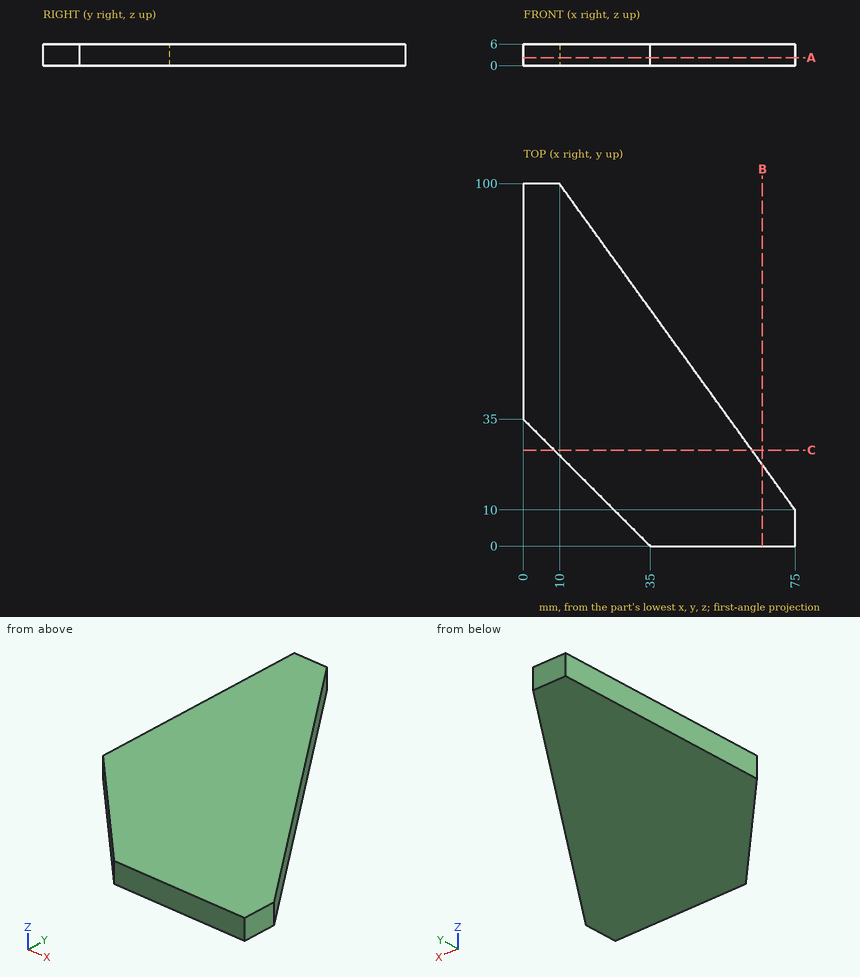
Could you check a few things on this drawing? It's one solid part, dimensions in mm from its lowest x, y, z. Round coordinates to 2 decimals unless told otherwise and drop trailing zeros. Loops run counter-clockwise (first coordinate to the right, second up) from the corner with the lowest first, then second, coordinate; pieces in that order, holes last. Notation, with made-up numbers: M -0.75,57 L 20.25,57 A28 cw 20.25,86 Z; hole C 1.5,84.25 d4. An arc over 180 degrees is marked long. Write each question's results on one line, items separated by ' | '. Start each with the question number.
(1) I want a section at A-A (z = 2.25). Please give me the cut outline in (x, y), then the cut area to 3 significant figures.
(2) Will these pins go through, and if not, where does the flat tip stop? P1, Ø2, axis at x = 30, z = 5, coming from the +Y side; P2, Ø3, axis at x = 25.5, y = 67.5, coming from the -Z side; P3, Ø1, axis at y = 83, z = 3.5, coming from the +X side; P4, Ø1.5, axis at x = 11, z = 0.5, coming from the +Y side.
(3) I want a section at C-C (y = 26.5). Please give me the cut outline in (x, z), then the cut area to 4 significant figures.
(4) If I drill on probe 1 along Y at (x, z) = (55, 2.25); probe 2 along X at (y, z) = (68, 2.5); probe 3 along X at (y, z) = (16, 4.5), over which ranges is the centre line in solid material (lowest first)? Write a range as from..to.
(5) I want a section at B-B (x = 66). Please give me the cut outline in (y, z), then the cut area to 3 significant figures.
Solved:
1) outline: M 0,35 L 35,0 L 75,0 L 75,10 L 10,100 L 0,100 Z | area: 3,960 mm²
2) P1: stops at y = 73.69 | P2: stops at z = 0 | P3: stops at x = 22.64 | P4: stops at y = 99.65
3) outline: M 8.5,0 L 63.08,0 L 63.08,6 L 8.5,6 Z | area: 327.5 mm²
4) probe 1: y = 0..37.69 | probe 2: x = 0..33.11 | probe 3: x = 19..70.67
5) outline: M 0,0 L 22.46,0 L 22.46,6 L 0,6 Z | area: 135 mm²
